```python
from build123d import *

# Parameters (mm, degrees)
EXTRUDE_1_DEPTH     = 6
CUT_EXTRUDE_1_DEPTH = 73.154348448
SKETCH_5_W          = 60
SKETCH_5_H          = 10
CUT_EXTRUDE_2_DEPTH = 1
CHAMFER_1_SIZE      = 1


with BuildPart() as part:
    # 草图1 → 凸台-拉伸1 (new, symmetric)
    with BuildSketch(Plane.XY):
        with BuildLine():
            Line((0, 0), (0, 4))
            Line((0, 4), (0.75, 3.566987298))
            ThreePointArc((0.75, 3.566987298), (3.25, 3.566987298), (4.5, 5.732050808))
            Line((4.5, 5.732050808), (4.5, 9.5))
            ThreePointArc((4.5, 9.5), (4.060660172, 10.560660172), (3, 11))
            Line((3, 11), (0, 11))
            Line((0, 11), (0, 20))
            Line((0, 20), (60, 20))
            Line((60, 20), (60, 1))
            Line((60, 1), (64, 1))
            Line((64, 1), (66, 3))
            Line((66, 3), (70, 3))
            Line((70, 3), (70, -24.5))
            Line((70, -24.5), (60, -24.5))
            Line((60, -24.5), (60, -38.357864376))
            Line((60, -38.357864376), (50, -42.5))
            Line((50, -42.5), (48, -42.5))
            Line((48, -42.5), (48, -24.5))
            Line((48, -24.5), (24, -24.5))
            Line((24, -24.5), (24, -38.357864376))
            Line((24, -38.357864376), (14, -42.5))
            Line((14, -42.5), (12, -42.5))
            Line((12, -42.5), (12, -1.5))
            Line((12, -1.5), (12.5, -1.5))
            Line((12.5, -1.5), (12.5, 0))
            Line((12.5, 0), (0, 0))
        make_face()
    extrude(amount=EXTRUDE_1_DEPTH, both=True)

    # 草图2 → 切除-拉伸1 (cut, through all)
    with BuildSketch(Plane.ZY.offset(-12)):
        Polygon((6, -25.705771366), (6, -47.5), (-6, -47.5), (-6, -25.705771366), (-1.5, -42.5), (1.5, -42.5), align=None)
    extrude(amount=-CUT_EXTRUDE_1_DEPTH, mode=Mode.SUBTRACT)

    # 草图5 → 切除-拉伸2 (cut)
    with BuildSketch(Plane(origin=(0, 20, 0), x_dir=(1, 0, 0), z_dir=(0, 1, 0))):
        with Locations((30, 0)):
            Rectangle(SKETCH_5_W, SKETCH_5_H)
    extrude(amount=-CUT_EXTRUDE_2_DEPTH, mode=Mode.SUBTRACT)

    # 倒角1
    chamfer_1_edges = [part.edges().sort_by_distance(p)[0] for p in [
        (70, -10.75, -6),
        (70, -10.75, 6),
    ]]
    chamfer(chamfer_1_edges, length=CHAMFER_1_SIZE)


solid = part.part
```
Geometry: final body of the model. Coordinates: model frame, mm. A direction names the side the tool comes from. Coordinates: 2 decimals unless noted, no trailing zeros. Order: outer loops, then holes, each group sorted by start corner. A loop starts at its lowest first (then second) coordinate and runs counter-clockwise, first axis right, second up. Notation, with made-up numbers: (-15, -7.5) -> (25, -7.5) arc R16 ccw to (25, 8.5) -> close; hole circle Ø8 at (82.25, 28). An arc over 180 degrees is marked (long way). Answer in a Markdown table with one row per item.
Item 1: Contact query for flat-ended pins moving along their axis: P1, Ø0.9, axis at x = 1, z = 2, coming from the -Y side; P2, Ø1.9, axis at y = 8.5, z = 2.5, coming from the -X side; P3, Ø1.6, axis at y = -1, z = 3, coming from the -X side. Output: stop coordinate, or through.
Return value:
| item | result |
|---|---|
| P1 | stops at y = 0 |
| P2 | stops at x = 4.5 |
| P3 | stops at x = 12 |
Item 2: Section C-C on y = -7.5. Output: boundary loops of the cut face in (x, z).
Return value:
| item | result |
|---|---|
| outline | (12, -6) -> (69, -6) -> (70, -5) -> (70, 5) -> (69, 6) -> (12, 6) -> close |
Item 3: Section B-B on x = 47. Output: boundary loops of the cut face in (y, z), plus the area to 3 significant figures.
Return value:
| item | result |
|---|---|
| outline | (-24.5, -6) -> (20, -6) -> (20, -5) -> (19, -5) -> (19, 5) -> (20, 5) -> (20, 6) -> (-24.5, 6) -> close |
| area | 524 mm² |
Item 4: Section D-D on z = -4. Output: boundary loops of the cut face in (x, y), plus the area to 3 significant figures.
Return value:
| item | result |
|---|---|
| outline | (0, 0) -> (12.5, 0) -> (12.5, -1.5) -> (12, -1.5) -> (12, -33.17) -> (24, -33.17) -> (24, -24.5) -> (48, -24.5) -> (48, -33.17) -> (60, -33.17) -> (60, -24.5) -> (70, -24.5) -> (70, 3) -> (66, 3) -> (64, 1) -> (60, 1) -> (60, 19) -> (0, 19) -> (0, 11) -> (3, 11) arc R1.5 cw to (4.5, 9.5) -> (4.5, 5.73) arc R2.5 cw to (0.75, 3.57) -> (0, 4) -> close |
| area | 2,760 mm² |
Item 5: Ray query, L1, parallel to X at y = -27, z = 4; L2, parallel to X at y = 12, z = 5.5; L3, parallel to X at y = -7, z = 0.75. Return the intervals inside material, ascending.
Return value:
| item | result |
|---|---|
| L1 | x = 12 to 24, 48 to 60 |
| L2 | x = 0 to 60 |
| L3 | x = 12 to 70 |
Item 6: Section A-A on z = 0.25. Output: boundary loops of the cut face in (x, y), plus the area to 3 significant figures.
Return value:
| item | result |
|---|---|
| outline | (0, 0) -> (12.5, 0) -> (12.5, -1.5) -> (12, -1.5) -> (12, -42.5) -> (14, -42.5) -> (24, -38.36) -> (24, -24.5) -> (48, -24.5) -> (48, -42.5) -> (50, -42.5) -> (60, -38.36) -> (60, -24.5) -> (70, -24.5) -> (70, 3) -> (66, 3) -> (64, 1) -> (60, 1) -> (60, 19) -> (0, 19) -> (0, 11) -> (3, 11) arc R1.5 cw to (4.5, 9.5) -> (4.5, 5.73) arc R2.5 cw to (0.75, 3.57) -> (0, 4) -> close |
| area | 2,940 mm² |
Item 7: Access query for faces 1 (the cylindrical face through (3.22, 3.55, 0.08)), 2 (the flat face through (68, 3, 0)), 3 (the cylindrical face through (4.07, 10.55, 0.08)), 4 (the flat face through (36, -24.5, 0)). Directions: +Z, -Z, +X, -X, +Y, -Y. A direction counts if a zero-diameter tool reaches every point of the face in a straight line with its end or side. Return the directions, or none.
Return value:
| item | result |
|---|---|
| face 1 | +Z, -Z |
| face 2 | +Z, -Z, +X, +Y |
| face 3 | +Z, -Z, -X |
| face 4 | +Z, -Z, -Y |
Item 8: Draft query along X for faces 5 (the flat face through (48, -32, 0)), 6 (the flat face through (30, 19, 0)), 7 (the flat face through (12, -18, 0)). Return one class per face: released by +X, released by -X, zero draft, split by the parting line, or undercut.
Return value:
| item | result |
|---|---|
| face 5 | undercut |
| face 6 | zero draft |
| face 7 | released by -X |
